Work out the finished part from the listing and answer in its coordinate system (mm). A direction names the side the tool comes from. Give positions to 0.01 mm unless a question says otherwise; leave off trailing zeros. Loops run counter-clockwise (first coordinate to the right, second up) from the corner with the lowest first, then second, coordinate; pieces in that order, holes last. Notation, with made-up numbers: (-21.5, 55) - (-17.5, 55) arc R8 ccw to (-17.5, 64) - close; hole circle Ø5 at (7, 27.25). An arc over 180 degrees is marked (long way). Use CSV: the item, a comma, the result in double quotes.
from build123d import *

# Parameters (mm, degrees)
SKETCH1_W              = 85
SKETCH1_H              = 15
EXTRUDE1_DEPTH         = 6
M12X1_0_TAPPED_HOLE1_D = 10.8
CHAMFER1_SIZE          = 2


with BuildPart() as part:
    # Sketch1 → Extrude1 (new body)
    with BuildSketch(Plane(origin=(0, 0, 0), x_dir=(0, 0, -1), z_dir=(1, 0, 0))):
        with Locations((42.5, -7.5)):
            Rectangle(SKETCH1_W, SKETCH1_H)
        with BuildLine():
            Line((22, -4.4), (77, -4.4))
            ThreePointArc((77, -4.4), (80.1, -7.5), (77, -10.6))
            Line((77, -10.6), (22, -10.6))
            ThreePointArc((22, -10.6), (18.9, -7.5), (22, -4.4))
        make_face(mode=Mode.SUBTRACT)
    extrude(amount=EXTRUDE1_DEPTH)

    # M12x1.0 Tapped Hole1 (through all)
    with Locations(Plane(origin=(6, 0, 0), x_dir=(0, 0, -1), z_dir=(1, 0, 0))):
        with Locations((7.5, -7.5)):
            Hole(M12X1_0_TAPPED_HOLE1_D / 2)

    # Chamfer1
    chamfer1_edges = [part.edges().sort_by_distance(p)[0] for p in [
        (3, 0, 0),
        (3, 0, -85),
        (3, -15, -85),
        (3, -15, 0),
    ]]
    chamfer(chamfer1_edges, length=CHAMFER1_SIZE)


solid = part.part
Item 1: Find the intervals of material crossed by line 1 (Z direction, x = 1.7, y = -7.25); line 2 (Y direction, x = 4.7, z = -54); line 3 (Z direction, x = 4.35, y = -10), in increasing order.
Determined:
line 1,"z = -85 to -80.09, -18.91 to -12.89, -2.11 to 0"
line 2,"y = -15 to -10.6, -4.4 to 0"
line 3,"z = -85 to -78.83, -20.17 to -12.29, -2.71 to 0"
Item 2: The mould has two halves that part along Z. Classify faces 1 (the flat face through (3, -1, -84)), 2 (the flat face through (6, -11, -42)), 3 (the cylindrical face through (3, -7.6, -18.9)), 4 (the flat face through (3, -10.6, -50)): pulls with the +Z half, pulls with the -Z half, needs draft (parallel to the pull), parting line crosses it, or undercut.
Determined:
face 1,"pulls with the -Z half"
face 2,"needs draft"
face 3,"undercut"
face 4,"undercut"
Item 3: For faces 5 (the flat face through (3, -8, -85)), 6 (the flat face through (3, -4.4, -49)), determine the directions among +Z, -Z, +X, -X, +Y, -Y from which every point of the face is accessible in a straight line to the end or side of a thin tool.
Determined:
face 5,"-Z, +X, -X, +Y, -Y"
face 6,"+X, -X"
Item 4: A cutting plane is placed at D-D on z = -7.5. Determine the outline of the cut face in (x, y), and give its area (3 significant figures).
Determined:
outline,"(0, -15) - (6, -15) - (6, -12.9) - (0, -12.9) - close; (0, -2.1) - (6, -2.1) - (6, 0) - (0, 0) - close"
area,"25.2 mm²"
Item 5: A cutting plane is placed at A-A on z = -23.5. Determine the outline of the cut face in (x, y), and give its area (3 significant figures).
Determined:
outline,"(0, -15) - (6, -15) - (6, -10.6) - (0, -10.6) - close; (0, -4.4) - (6, -4.4) - (6, 0) - (0, 0) - close"
area,"52.8 mm²"
Item 6: A cutting plane is placed at C-C on y = -7.5. Determine the outline of the cut face in (x, z).
Determined:
outline,"(0, -85) - (6, -85) - (6, -80.1) - (0, -80.1) - close; (0, -18.9) - (6, -18.9) - (6, -12.9) - (0, -12.9) - close; (0, -2.1) - (6, -2.1) - (6, 0) - (0, 0) - close"
Item 7: A cutting plane is placed at B-B on x = 1.6. Determine the outline of the cut face in (y, z), and give its area (3 significant figures).
Determined:
outline,"(-15, -83) - (-13, -85) - (-2, -85) - (0, -83) - (0, -2) - (-2, 0) - (-13, 0) - (-15, -2) - close; hole circle Ø10.8 at (-7.5, -7.5); hole (-10.6, -77) arc R3.1 ccw to (-4.4, -77) - (-4.4, -22) arc R3.1 ccw to (-10.6, -22) - close"
area,"804 mm²"
